Work out the finished part from the listing and answer in its coordinate system (mm). A direction names the side the tool comes from. Coordinates: 2 decimals unless noted, no trailing zeros. Order: outer loops, then holes, each group sorted by start corner. A loop starts at its lowest first (then second) coordinate and runs counter-clockwise, first axis right, second up.
1. Find the intervals of material crossed by probe 1 along Y at (x, z) = (-30.5, 85); probe 2 along Z at (x, y) = (-35.5, 87.5); probe 3 along X at (y, z) = (67, -2), in increasing order.
2. Determine the mould class of faces 5 (the cylindrical face through (-8.87, 15.62, -3.47)), 6 (the flat face through (-44, 68, 0)), 7 (the flat face through (0, -12, -12)), 8 (the cylindrical face through (-8.87, -24.84, -12.92)) for opening direction Y: +Y half, -Y half, draft (parallel to the pull), parting line (faces both ways), or undercut.
3. The part is cut by section B-B, the plane y = 10. Give the vertices of the cut face in (x, z).
4. The part is cut by section C-C, the plane x = -7.5. Give the vertices of the cut face in (y, z).
5. A tool of negligible diameter and unlimited length cuts with its end or side. For faces 1 (the flat face through (-4, 33, 0)), 2 (the flat face through (-46, 117, 67)), 3 (the flat face through (-55, 40, 0)), 4 (the flat face through (-61, 117, 55)), from which of +Z, -Z, +X, -X, +Y, -Y can it reach the whole face along a straight path? Write none if from no direction.
6. The part is cut by section A-A, the plane x = -59. Give the vertices of the cut face in (y, z), then the cut area to 3 significant figures.
7. Flat-ended cylindrical pins translate along their axes: pin 1 Ø21 at (x, z) = (-48, 47.5) entering from -Y; pin 2 Ø18 at (y, z) = (116, 30.5) entering from -X; pin 3 Ø6 at (x, y) = (-29, 78) entering from -Z; pin 4 Ø9 at (y, z) = (117, 85) entering from +X. Find the tip coordinate at first contact, or state that the pin passes through.
8. The part is cut by section D-D, the plane z = 30.5. Give the vertices of the cut face in (x, y).
```python
from build123d import *

# Parameters (mm, degrees)
LOWER_HUB_A_SKETCH_R        = 28
LOWER_HUB_A_56_DEPTH        = 18
LOWER_HUB_B_SKETCH_R        = 28
LOWER_HUB_B_56_DEPTH        = 18
LOWER_FORK_BLOCK_DEPTH      = 48
LOWER_FORK_BLOCK_DEPTH_BACK = 14
LOWER_FORK_SLOT_SKETCH_W    = 34
LOWER_FORK_SLOT_SKETCH_H    = 15.390479787
LOWER_FORK_SLOT_DEPTH       = 65
VERTICAL_ARM_DEPTH          = 50
UPPER_HUB_DEPTH             = 3
UPPER_HUB_DEPTH_BACK        = 43
UPPER_HUB_SKETCH_R          = 25
UPPER_FORK_ARM_DEPTH        = 36
FORK_EYE_A_SKETCH_R         = 18
FORK_EYE_A_36_DEPTH         = 15
FORK_START                  = -15
FORK_EYE_B_SKETCH_R         = 18
FORK_EYE_B_DEPTH            = 15
LOWER_PIVOT_BORE_SKETCH_R   = 16
LOWER_PIVOT_BORE_32_DEPTH   = 132
UPPER_HUB_BORE_SKETCH_R     = 12.5
UPPER_HUB_BORE_25_DEPTH     = 132
FORK_EYE_BORE_SKETCH_R      = 7.5
FORK_EYE_BORE_15_DEPTH      = 132


with BuildPart() as part:
    # Lower Hub A Sketch → Lower Hub A Ø56 (new body)
    with BuildSketch(Plane(origin=(0, 0, 0), x_dir=(0, 0, -1), z_dir=(1, 0, 0))):
        Circle(LOWER_HUB_A_SKETCH_R)
    extrude(amount=-LOWER_HUB_A_56_DEPTH)



with BuildPart() as body_2:
    # Lower Hub B Sketch → Lower Hub B Ø56 (new body)
    with BuildSketch(Plane.ZY.offset(52)):
        with Locations(Location((0, 0, 0), (0, 0, 180))):
            Circle(LOWER_HUB_B_SKETCH_R)
    extrude(amount=LOWER_HUB_B_56_DEPTH)


with BuildPart() as part_1:
    add(part.part)

    add(body_2.part)  # Lower Fork Block merges body 2
    # Lower Fork Block Sketch → Lower Fork Block (add, two sides: drawn at the far end of the back side and taken through both)
    with BuildSketch(Plane.ZY.offset(18).offset(-LOWER_FORK_BLOCK_DEPTH_BACK)):
        with BuildLine():
            Line((0, 40), (25, 40))
            Line((25, 40), (25, 12.609520213))
            ThreePointArc((25, 12.609520213), (0, 28), (-25, 12.609520213))
            Line((-25, 12.609520213), (-25, 40))
            Line((-25, 40), (0, 40))
        make_face()
    extrude(amount=LOWER_FORK_BLOCK_DEPTH + LOWER_FORK_BLOCK_DEPTH_BACK)

    # Lower Fork Slot Sketch → Lower Fork Slot (cut)
    with BuildSketch(Plane.XY.offset(25)):
        with Locations((-35, 20.304760107)):
            Rectangle(LOWER_FORK_SLOT_SKETCH_W, LOWER_FORK_SLOT_SKETCH_H)
    extrude(amount=-LOWER_FORK_SLOT_DEPTH, mode=Mode.SUBTRACT)

    # Vertical Arm Sketch → Vertical Arm (add)
    with BuildSketch(Plane.XY.offset(25)):
        Polygon((-35, 40), (-26, 40), (-26, 110), (-44, 110), (-44, 40), align=None)
    extrude(amount=-VERTICAL_ARM_DEPTH)

    # Upper Hub Sketch → Upper Hub (add, two sides: drawn at the far end of the back side and taken through both)
    with BuildSketch(Plane(origin=(-26, 0, 0), x_dir=(0, 0, -1), z_dir=(1, 0, 0)).offset(-UPPER_HUB_DEPTH_BACK)):
        with Locations((0, 110)):
            Circle(UPPER_HUB_SKETCH_R)
    extrude(amount=UPPER_HUB_DEPTH + UPPER_HUB_DEPTH_BACK)

    # Upper Fork Arm Sketch → Upper Fork Arm (add)
    with BuildSketch(Plane(origin=(0, 135, 0), x_dir=(1, 0, 0), z_dir=(0, 1, 0))):
        Polygon((-37, 0), (-37, -55), (-25, -55), (-25, -85), (-37, -85), (-37, -67), (-55, -67), (-55, -85), (-67, -85), (-67, -55), (-55, -55), (-55, 0), align=None)
    extrude(amount=-UPPER_FORK_ARM_DEPTH)

    # Fork Eye A Sketch → Fork Eye A Ø36 (add)
    with BuildSketch(Plane(origin=(-55, 0, 0), x_dir=(0, 0, -1), z_dir=(1, 0, 0))):
        with Locations((-85, 117)):
            Circle(FORK_EYE_A_SKETCH_R)
    extrude(amount=-FORK_EYE_A_36_DEPTH)

    # Fork Eye B Sketch → Fork Eye B (add)
    with BuildSketch(Plane.ZY.offset(37).offset(FORK_START)):
        with Locations(Location((85, 117, 0), (0, 0, 180))):
            Circle(FORK_EYE_B_SKETCH_R)
    extrude(amount=FORK_EYE_B_DEPTH)

    # Lower Pivot Bore Sketch → Lower Pivot Bore Ø32 (cut)
    with BuildSketch(Plane(origin=(0, 0, 0), x_dir=(0, 0, -1), z_dir=(1, 0, 0))):
        with Locations(Location((0, 0, 0), (0, 0, 180))):
            Circle(LOWER_PIVOT_BORE_SKETCH_R)
    extrude(amount=-LOWER_PIVOT_BORE_32_DEPTH, mode=Mode.SUBTRACT)

    # Upper Hub Bore Sketch → Upper Hub Bore Ø25 (cut)
    with BuildSketch(Plane.ZY.offset(69)):
        with Locations((0, 110)):
            Circle(UPPER_HUB_BORE_SKETCH_R)
    extrude(amount=-UPPER_HUB_BORE_25_DEPTH, mode=Mode.SUBTRACT)

    # Fork Eye Bore Sketch → Fork Eye Bore Ø15 (cut)
    with BuildSketch(Plane.ZY.offset(70)):
        with Locations((85, 117)):
            Circle(FORK_EYE_BORE_SKETCH_R)
    extrude(amount=-FORK_EYE_BORE_15_DEPTH, mode=Mode.SUBTRACT)


solid = part_1.part
```
Geometry says:
1. probe 1: y = 99 to 109.5, 124.5 to 135
1. probe 2: z = -25 to 25
1. probe 3: x = -44 to -26
2. face 5: undercut
2. face 6: undercut
2. face 7: draft
2. face 8: parting line
3. outline: (-70, -26.15) - (-52, -26.15) - (-52, -12.49) - (-70, -12.49) - close; (-70, 12.49) - (-52, 12.49) - (-52, 26.15) - (-70, 26.15) - close; (-18, -26.15) - (0, -26.15) - (0, -12.49) - (-18, -12.49) - close; (-18, 12.49) - (0, 12.49) - (0, 26.15) - (-18, 26.15) - close
4. outline: (12.61, -25) - (40, -25) - (40, 25) - (12.61, 25) arc R28 ccw (long way) to start; hole circle Ø32 at (0, 0)
5. face 1: +X, +Y
5. face 2: +Z, +Y, -Y
5. face 3: +Z, -Z, -X
5. face 4: -X, +Y, -Y
6. outline: (12.61, -25) - (40, -25) - (40, 25) - (12.61, 25) arc R28 ccw (long way) to start; circle Ø50 at (110, 0); (99, 55) - (135, 55) - (135, 85) arc R18 ccw to (99, 85) - close; hole circle Ø32 at (0, 0); hole circle Ø25 at (110, 0); hole circle Ø15 at (117, 85)
6. area: 5,360 mm2
7. pin 1: stops at y = 99
7. pin 2: stops at x = -69
7. pin 3: stops at z = -25
7. pin 4: passes through
8. outline: (-55, 99) - (-37, 99) - (-37, 135) - (-55, 135) - close
